Geometry check sheet. Reference: the model listing, model coordinates, mm. A direction names the side the tool comes from. Coordinates: 2 decimals unless noted, no trailing zeros. Order: outer loops, then holes, each group sorted by start corner. A loop starts at its lowest first (then second) coordinate and runs counter-clockwise, first axis right, second up. Notation, with made-up numbers: M -10.75,-16 L 13.25,-16 A28 cw 13.25,15 Z; hole C 27.25,-13.75 d5. An arc over 180 degrees is marked long. One line per item, written item: value. Start each with the question number.
1) Access from +Z, -Z, +X, -X, +Y, -Y to the whole of each face (thin tool, end or side, straight path). Record for faces 3 (the flat face through (-12.7, -82, 16)), 4 (the flat face through (-88.468, -59, 38)), 5 (the flat face through (-54, 77.724, 0)).
2) Sectioned sample at A-A, the plane z = 95.25. Enter the section's corners in (x, y), then the cut area to 3 significant figures.
3) Sectioned sample at D-D, the plane x = -37. Enter the section's corners in (y, z).
4) Sectioned sample at C-C, the plane y = 0. State how many separate pieces and enclosed holes the cut face has, then the cut area to 3 significant figures.
5) Go/stop test with flat-tipped pins: P1, Ø23, axis at y = 61.22, z = 72.97, coming from the +X side; P2, Ø23, axis at y = -82.5, z = 47.62, coming from the -X side; P3, Ø6, axis at x = -18.5, z = 70.5, coming from the +Y side; P4, Ø2, axis at x = -76, y = -41.5, coming from the +Z side. Record where each tip stops, or that it passes through.
6) Thickness scan on L1, parallel to Z at x = -90, y = 0; L2, parallel to Z at x = -65, y = 0; L3, parallel to X at y = 26.5, z = -61. Record the ranges inside material, lowest first. Write a range as from..to.
7) Draft check along Z on faces 1 (the flat face through (-95.25, -36, -61)), 2 (the cylindrical face through (-32.266, -8.581, -65.352)). Enter one of: pulls with the +Z half, pulls with the -Z half, needs draft (parallel to the pull), parting line crosses it, or undercut.
```python
from build123d import *

# Parameters (mm, degrees)
F_9_16_0_5625_DIAMETER_HOLE1_D = 14.2875
F_1_2_13_TAPPED_HOLE1_D        = 10.71626
EXTRUDE1_START                 = 77.724
SKETCH8_W                      = 58.674
SKETCH8_H                      = 38.1
EXTRUDE1_DEPTH                 = 4.8133
EXTRUDE2_REACH                 = 240.925
EXTRUDE2_END_RADIUS            = 65.913
SKETCH9_R                      = 9.525
FILLET1_R                      = 3
EXTRUDE3_REACH                 = 185.766


with BuildPart() as part:
    # Sketch1 → Revolve1 (revolve)
    with BuildSketch(Plane.XY):
        Polygon((-95.25, 70.620031854), (-95.25, 82.2956), (-88.9, 82.5373), (-12.7, 82.5373), (-12.7, 111.125), (0, 111.125), (0, 0), (-24.2804, 0), (-24.2804, 65.913), (-40.0304, 65.913), (-40.0304, 70.0075), (-88.4682, 70.0075), (-88.4682, 73.279), (-91.5162, 73.279), (-91.5162, 70.0075), (-92.964, 70.0075), align=None)
    revolve(axis=Axis((0, 0, 0), (-1, 0, 0)))

    # 9/16 (0.5625) Diameter Hole1 (through all)
    with Locations(Plane(origin=(0, 0, 0), x_dir=(0, 0, -1), z_dir=(1, 0, 0))):
        with Locations((-72.9742, 61.2154), (72.9742, 61.2154), (-47.625, -82.4992), (47.625, -82.4992)):
            Hole(F_9_16_0_5625_DIAMETER_HOLE1_D / 2)

    # 1/2-13 Tapped Hole1 (through all)
    with Locations(Plane(origin=(0, 0, 0), x_dir=(0, 0, -1), z_dir=(1, 0, 0))):
        with Locations((-95.25, 0), (95.25, 0)):
            Hole(F_1_2_13_TAPPED_HOLE1_D / 2)

    # Sketch8 → Extrude1 (cut)
    with BuildSketch(Plane(origin=(0, 0, 0), x_dir=(1, 0, 0), z_dir=(0, 1, 0)).offset(EXTRUDE1_START)):
        with Locations((-53.6174, 0)):
            Rectangle(SKETCH8_W, SKETCH8_H)
    extrude(amount=EXTRUDE1_DEPTH, mode=Mode.SUBTRACT)

    # Extrude2: up to this cylinder (the profile starts outside it)
    extrude2_end = Plane(origin=(-33.8054, 0, 0), z_dir=(1, 0, 0)) * Cylinder(EXTRUDE2_END_RADIUS, 614.676, mode=Mode.PRIVATE)
    # Sketch9 → Extrude2 (cut, up to the surface)
    with BuildSketch(Plane(origin=(0, 77.724, 0), x_dir=(1, 0, 0), z_dir=(0, 1, 0)), mode=Mode.PRIVATE) as extrude2_sk1:
        with Locations((-33.8054, 0)):
            Circle(SKETCH9_R)
    extrude2_tool1 = extrude(extrude2_sk1.sketch, amount=-EXTRUDE2_REACH, mode=Mode.PRIVATE) - extrude2_end
    add(extrude2_tool1.solids().sort_by_distance((-33.8054, 77.724, 0))[0], mode=Mode.SUBTRACT)

    # Fillet1
    fillet1_edges = [part.edges().sort_by_distance(p)[0] for p in [
        (-82.9544, 79.016400105, 19.05),
        (-82.9544, 79.016400105, -19.05),
    ]]
    fillet(fillet1_edges, radius=FILLET1_R)

    # Sketch10 → Extrude3 (cut, up to next)
    with BuildSketch(Plane(origin=(0, 0, 0), x_dir=(0, 0, -1), z_dir=(1, 0, 0)), mode=Mode.PRIVATE) as extrude3_sk1:
        with BuildLine():
            ThreePointArc((-15.708416989, 110.009141714), (0, 95.377), (15.708416989, 110.009141714))
            ThreePointArc((15.708416989, 110.009141714), (0, 111.125), (-15.708416989, 110.009141714))
        make_face()
    extrude3_tool1 = extrude(extrude3_sk1.sketch, amount=-EXTRUDE3_REACH, mode=Mode.PRIVATE) & part.part
    add(extrude3_tool1.solids().sort_by_distance((0, 104.244395, 0))[0], mode=Mode.SUBTRACT)


solid = part.part
```
Final values:
1. face 3: -X
1. face 4: none
1. face 5: +Y
2. outline: M -12.7,-57.24 L 0,-57.24 L 0,-5.36 L -12.7,-5.36 Z; M -12.7,5.36 L 0,5.36 L 0,57.24 L -12.7,57.24 Z
2. area: 1,320 mm^2
3. outline: M 65.3,-8.97 A65.91 cw long 65.3,8.97 L 77.72,8.97 L 77.72,19.05 L 80.31,19.05 A82.54 ccw long 80.31,-19.05 L 77.72,-19.05 L 77.72,-8.97 Z
4. separate pieces: 3
4. enclosed holes: 0
4. area: 6,350 mm^2
5. P1: stops at x = 0
5. P2: stops at x = -12.7
5. P3: stops at y = 47.5
5. P4: stops at z = 71.92
6. L1: z = -82.5..-73.28, 73.28..82.5
6. L2: z = -82.54..-70.01, 70.01..82.54
6. L3: x = -40.03..0
7. face 1: needs draft
7. face 2: undercut
